Part model, mm, in its own coordinate system. A direction names the side the tool comes from. Round coordinates to 2 decimals unless told otherwise and drop trailing zeros. Write each loop counter-clockwise with the first axis right and the second up, starting at its lowest first coordinate (ties: lowest second). Pieces come first, ordered by that corner, then holes. Notation, with made-up numbers: (-7, -5) -> (22, -5) arc R23 cw to (22, 22) -> close; hole circle Ø11 at (-22.75, 40.25). An arc over 180 degrees is marked (long way). Return JSON: item names as keys, results as strings. Group by question number.
```python
from build123d import *

# Parameters (mm, degrees)
FLANGE_PROFILE_SKETCH_R = 17
FLANGE_34X4_DEPTH       = 4
HUB_PROFILE_SKETCH_R    = 6.25
HUB_PROFILE_SKETCH_R_2  = 4
HUB_TUBE_20MM_DEPTH     = 20
BOLT_HOLES_SKETCH_R     = 2
BOLT_HOLES_4X_DEPTH     = 4
REAR_START              = 1
REAR_SPIGOT_SKETCH_R    = 6.25
REAR_SPIGOT_SKETCH_R_2  = 4
REAR_SPIGOT_1MM_DEPTH   = 1


with BuildPart() as part:
    # Flange Profile Sketch → Flange Ø34x4 (new body)
    with BuildSketch(Plane.XY):
        Circle(FLANGE_PROFILE_SKETCH_R)
    extrude(amount=FLANGE_34X4_DEPTH)

    # Hub Profile Sketch → Hub Tube 20mm (add)
    with BuildSketch(Plane.XY.offset(4)):
        Circle(HUB_PROFILE_SKETCH_R)
        Circle(HUB_PROFILE_SKETCH_R_2, mode=Mode.SUBTRACT)
    extrude(amount=HUB_TUBE_20MM_DEPTH)

    # Bolt Holes Sketch → Bolt Holes 4x (cut)
    with BuildSketch(Plane.XY.offset(4)):
        with Locations((0, 12.5)):
            Circle(BOLT_HOLES_SKETCH_R)
        with Locations((12.5, 0)):
            Circle(BOLT_HOLES_SKETCH_R)
        with Locations((0, -12.5)):
            Circle(BOLT_HOLES_SKETCH_R)
        with Locations((-12.5, 0)):
            Circle(BOLT_HOLES_SKETCH_R)
    extrude(amount=-BOLT_HOLES_4X_DEPTH, mode=Mode.SUBTRACT)

    # Rear Spigot Sketch → Rear Spigot 1mm (add)
    with BuildSketch(Plane(origin=(0, 0, 0), x_dir=(-1, 0, 0), z_dir=(0, 0, -1)).offset(REAR_START)):
        with Locations(Location((0, 0, 0), (0, 0, 180))):
            Circle(REAR_SPIGOT_SKETCH_R)
        with Locations(Location((0, 0, 0), (0, 0, 180))):
            Circle(REAR_SPIGOT_SKETCH_R_2, mode=Mode.SUBTRACT)
    extrude(amount=-REAR_SPIGOT_1MM_DEPTH)


solid = part.part
```
Item 1: Flat gauge pins, fed straight in: P1, Ø5, axis at x = 0, y = 0, coming from the +Z side; P2, Ø6.5, axis at x = 12.5, y = 0, coming from the -Z side; P3, Ø1, axis at y = 2.5, z = 19, coming from the +X side; P4, Ø10, axis at x = -1.5, z = 1.5, coming from the -Y side. Where does each tip first touch, or does it go through?
Item 2: Wall check: L1, parallel to Y at x = 0, z = 2.45; L2, parallel to Z at x = 10, y = 3.5; L3, parallel to Y at x = -1.5, z = 21. Give the ranges that are in metal, low to high.
Item 3: Which spindle directions (+Z, -Z, +X, -X, +Y, -Y) get a long thin tool onto all of the face, cutting with end or side? Do faces 1 (the face through (7, 0, 4)), 2 (the face through (0, 0, 0)), 3 (the face through (1.3, 4.1, -1)). Say none if no direction does.
Item 4: Cut at C-C (x = -12.5). Write the cut outline in (y, z).
Item 5: Cut at A-A (y = 0). Write the cut outline in (x, z), then the cut area to 4 significant figures.
Item 6: Two-plate mould, pull along Y, no slides. Class faces 4 (the face through (1.3, -4.1, 24)), 5 (the face through (-0.26, 14.483, 2.028)), 6 (the face through (5.96, -1.88, -0.51)): released by +Y, released by -Y, zero draft, split by the parting line, or undercut.
Checks:
{
 "1": {"P1": "stops at z = 4", "P2": "stops at z = 0", "P3": "stops at x = 5.92", "P4": "stops at y = -17"},
 "2": {"L1": "y = -17 to -14.5, -10.5 to 10.5, 14.5 to 17", "L2": "z = 0 to 4", "L3": "y = -6.07 to -3.71, 3.71 to 6.07"},
 "3": {"face 1": "+Z", "face 2": "-Z", "face 3": "-Z, +X, -X, +Y, -Y"},
 "4": {"outline": "(-11.52, 0) -> (-2, 0) -> (-2, 4) -> (-11.52, 4) -> close; (2, 0) -> (11.52, 0) -> (11.52, 4) -> (2, 4) -> close"},
 "5": {"outline": "(-17, 0) -> (-14.5, 0) -> (-14.5, 4) -> (-17, 4) -> close; (-10.5, 0) -> (-6.25, 0) -> (-6.25, -1) -> (-4, -1) -> (-4, 0) -> (4, 0) -> (4, -1) -> (6.25, -1) -> (6.25, 0) -> (10.5, 0) -> (10.5, 4) -> (6.25, 4) -> (6.25, 24) -> (4, 24) -> (4, 4) -> (-4, 4) -> (-4, 24) -> (-6.25, 24) -> (-6.25, 4) -> (-10.5, 4) -> close; (14.5, 0) -> (17, 0) -> (17, 4) -> (14.5, 4) -> close", "area": "198.5 mm2"},
 "6": {"face 4": "zero draft", "face 5": "undercut", "face 6": "split by the parting line"}
}
